Verification items for the finished model (mm, model axes). Face numbers are marked on the shaded views. Give positions to 0.01 mm unless a question says otherwise; leave off trailing zeros. Write each loop counter-clockwise with the first axis right and the second up, starting at its lowest first coordinate (ties: lowest second). Pieces come first, ordered by that corner, then holes. Notation, with made-up numbers: (-31.5, -34) -> (20.5, -34) arc R20 ccw to (20.5, -1) -> close; hole circle Ø11 at (-23.75, 82). An arc over 180 degrees is marked (long way). Answer as CSV lines item,"result".
```python
from build123d import *

# Parameters (mm, degrees)
SKETCH1_R           = 2.6035
BOSS_EXTRUDE1_DEPTH = 9.652


with BuildPart() as part:
    # Sketch1 → Boss-Extrude1 (new body)
    with BuildSketch(Plane.XY):
        with BuildLine():
            Line((12.356395011, -0.759834892), (37.258046093, 28.076215001))
            ThreePointArc((37.258046093, 28.076215001), (42.63181619, 28.469654882), (43.025256071, 23.095884784))
            Line((43.025256071, 23.095884784), (18.123604989, -5.740165108))
            ThreePointArc((18.123604989, -5.740165108), (12.749834892, -6.133604989), (12.356395011, -0.759834892))
        make_face()
        with Locations(Location((15.24, -3.25, 0), (0, 0, 90))):
            Circle(SKETCH1_R, mode=Mode.SUBTRACT)
        with Locations(Location((40.141651082, 25.586049892, 0), (0, 0, 90))):
            Circle(SKETCH1_R, mode=Mode.SUBTRACT)
    extrude(amount=BOSS_EXTRUDE1_DEPTH)


solid = part.part
```
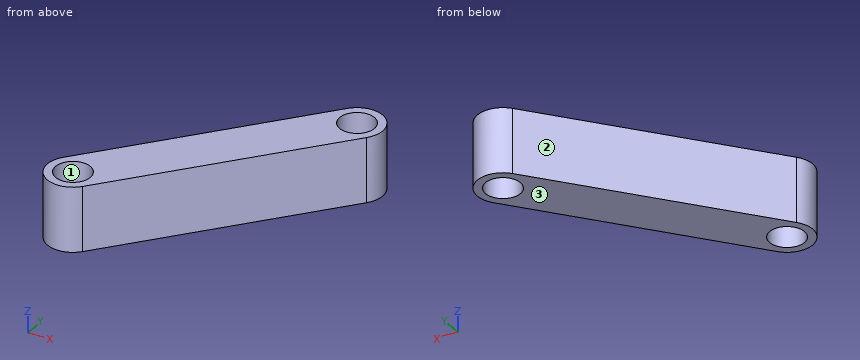
1) Section check B-B (y = -3.25). Record the boundary of the cut face in (x, z).
Reported:
outline,"(11.43, 0) -> (12.64, 0) -> (12.64, 9.65) -> (11.43, 9.65) -> close; (17.84, 0) -> (20.27, 0) -> (20.27, 9.65) -> (17.84, 9.65) -> close"
2) Scan lines: line 1 along X through (y, z) = (26, 4.25); line 2 along X through (y, z) = (-3.25, 2.75); line 3 along Y through (x, z) = (15.24, 4). Record each from-to range of solid material in increasing order.
Reported:
line 1,"35.47 to 37.57, 42.71 to 43.93"
line 2,"11.43 to 12.64, 17.84 to 20.27"
line 3,"-7.06 to -5.85, -0.65 to 2.58"
3) Section check A-A (x = 15.24). Record the boundary of the cut face in (y, z), and give its area (3 significant figures).
Reported:
outline,"(-7.06, 0) -> (-5.85, 0) -> (-5.85, 9.65) -> (-7.06, 9.65) -> close; (-0.65, 0) -> (2.58, 0) -> (2.58, 9.65) -> (-0.65, 9.65) -> close"
area,"42.8 mm²"
4) Draft check along X on the marked faces 1, 2 and 3. Enter one of: +X half, -X half, draft (parallel to the pull), parting line (faces both ways), or undercut.
Reported:
face 1,"undercut"
face 2,"-X half"
face 3,"draft"
5) Section check C-C (z = 5.5). Record the boundary of the cut face in (x, y).
Reported:
outline,"(12.36, -0.76) arc R3.81 ccw to (18.12, -5.74) -> (43.03, 23.1) arc R3.81 ccw to (37.26, 28.08) -> close; hole circle Ø5.21 at (15.24, -3.25); hole circle Ø5.21 at (40.14, 25.59)"
6) Depth check by flat-ended pin: pin 1 (5 mm diameter, centred on y = 22, z = 6, fed in from -X); pin 2 (1.5 mm diameter, centred on x = 27, z = 5, fed in from -Y); pin 3 (4 mm diameter, centred on x = 40.5, z = 5.5, fed in from +Y); pin 4 (2 mm diameter, centred on x = 38, z = 4.5, fed in from +Y). Enter the tip coordinate at first touch or a pass-through.
Reported:
pin 1,"x = 29.85"
pin 2,"y = 3.67"
pin 3,"y = 29.4"
pin 4,"y = 29.22"
7) Section check D-D (x = 27). Record the boundary of the cut face in (y, z), and give its area (3 significant figures).
Reported:
outline,"(4.54, 0) -> (16.2, 0) -> (16.2, 9.65) -> (4.54, 9.65) -> close"
area,"113 mm²"
